Part model, mm, in its own coordinate system. Round coordinates to 2 decimals unless told otherwise and drop trailing zeros. Loops run counter-clockwise (first coordinate to the right, second up) from the corner with the lowest first, then second, coordinate; pieces in that order, holes last.
1) Band-saw the part on C-C, the plane y = 0.85. Write the cut outline in (x, z).
2) Band-saw the part on D-D, the plane z = 0. Write the cut outline in (x, y).
3) Probe line 1 (X direction, y = 0.7, z = -32.5); line 2 (X direction, y = 1.4, z = 31.5); line 3 (X direction, y = 1.3, z = 0). List the from-to ranges inside material, lowest first.
4) Band-saw the part on A-A, the plane z = 32.5. Write the cut outline in (x, y).
5) Band-saw the part on B-B, the plane x = 32.5. Write the cut outline in (y, z), then the cut area to 3 significant figures.
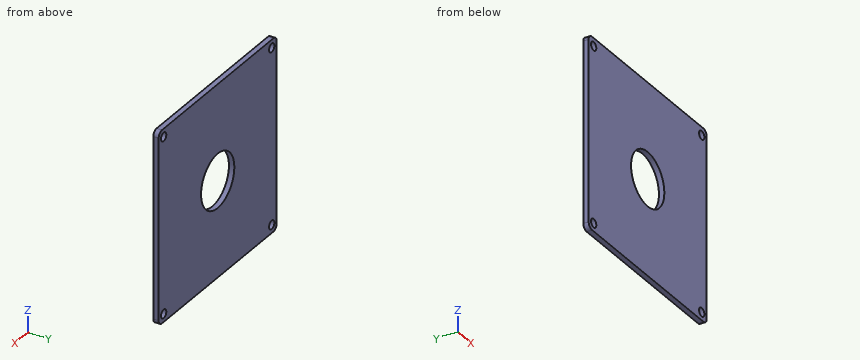
from build123d import *

# Parameters (mm, degrees)
SKETCH1_R           = 1.6
BOSS_EXTRUDE1_DEPTH = 2
SKETCH2_R           = 10
CUT_EXTRUDE1_DEPTH  = 10


with BuildPart() as part:
    # Sketch1 → Boss-Extrude1 (new body)
    with BuildSketch(Plane(origin=(0, 0, 0), x_dir=(1, 0, 0), z_dir=(0, 1, 0))):
        with BuildLine():
            Line((-33.5, -35.5), (33.5, -35.5))
            ThreePointArc((33.5, -35.5), (34.914213562, -34.914213562), (35.5, -33.5))
            Line((35.5, -33.5), (35.5, 33.5))
            ThreePointArc((35.5, 33.5), (34.914213562, 34.914213562), (33.5, 35.5))
            Line((33.5, 35.5), (-33.5, 35.5))
            ThreePointArc((-33.5, 35.5), (-34.914213562, 34.914213562), (-35.5, 33.5))
            Line((-35.5, 33.5), (-35.5, -33.5))
            ThreePointArc((-35.5, -33.5), (-34.914213562, -34.914213562), (-33.5, -35.5))
        make_face()
        with Locations(Location((-32.5, 32.5, 0), (0, 0, 270))):
            Circle(SKETCH1_R, mode=Mode.SUBTRACT)
        with Locations(Location((32.5, 32.5, 0), (0, 0, 270))):
            Circle(SKETCH1_R, mode=Mode.SUBTRACT)
        with Locations(Location((32.5, -32.5, 0), (0, 0, 270))):
            Circle(SKETCH1_R, mode=Mode.SUBTRACT)
        with Locations(Location((-32.5, -32.5, 0), (0, 0, 270))):
            Circle(SKETCH1_R, mode=Mode.SUBTRACT)
    extrude(amount=BOSS_EXTRUDE1_DEPTH)

    # Sketch2 → Cut-Extrude1 (cut)
    with BuildSketch(Plane(origin=(0, 2, 0), x_dir=(1, 0, 0), z_dir=(0, 1, 0))):
        with Locations(Location((0, 0, 0), (0, 0, 270))):
            Circle(SKETCH2_R)
    extrude(amount=-CUT_EXTRUDE1_DEPTH, mode=Mode.SUBTRACT)


solid = part.part
Reported:
1. outline: (-35.5, -33.5) arc R2 ccw to (-33.5, -35.5) - (33.5, -35.5) arc R2 ccw to (35.5, -33.5) - (35.5, 33.5) arc R2 ccw to (33.5, 35.5) - (-33.5, 35.5) arc R2 ccw to (-35.5, 33.5) - close; hole circle Ø3.2 at (-32.5, -32.5); hole circle Ø3.2 at (-32.5, 32.5); hole circle Ø20 at (0, 0); hole circle Ø3.2 at (32.5, -32.5); hole circle Ø3.2 at (32.5, 32.5)
2. outline: (-35.5, 0) - (-10, 0) - (-10, 2) - (-35.5, 2) - close; (10, 0) - (35.5, 0) - (35.5, 2) - (10, 2) - close
3. line 1: x = -35.5 to -34.1, -30.9 to 30.9, 34.1 to 35.5
3. line 2: x = -35.5 to -33.75, -31.25 to 31.25, 33.75 to 35.5
3. line 3: x = -35.5 to -10, 10 to 35.5
4. outline: (-35.5, 0) - (-34.1, 0) - (-34.1, 2) - (-35.5, 2) - close; (-30.9, 0) - (30.9, 0) - (30.9, 2) - (-30.9, 2) - close; (34.1, 0) - (35.5, 0) - (35.5, 2) - (34.1, 2) - close
5. outline: (0, -35.5) - (2, -35.5) - (2, -34.1) - (0, -34.1) - close; (0, -30.9) - (2, -30.9) - (2, 30.9) - (0, 30.9) - close; (0, 34.1) - (2, 34.1) - (2, 35.5) - (0, 35.5) - close
5. area: 129 mm2
